Build history of the part. All positions in model axes, mm. Round coordinates to 2 decimals unless told otherwise and drop trailing zeros. Loops run counter-clockwise (first coordinate to the right, second up) from the corner with the lowest first, then second, coordinate; pieces in that order, holes last. Notation, with made-up numbers: (-21, -2) - (-12, -2) arc R15 cw to (-12, 2) - close; hole circle Ø7 at (-7, 43.25). An arc over 180 degrees is marked (long way). Put each result on its own line as item: value. Start each with the question number.
from build123d import *

# Parameters (mm, degrees)
SKETCH_1_R      = 5
EXTRUDE_1_DEPTH = 185
SKETCH_2_R      = 4
EXTRUDE_2_DEPTH = 8
CHAMFER_1_SIZE  = 0.5


with BuildPart() as part:
    # 草图1 → 凸台-拉伸1 (new body)
    with BuildSketch(Plane.XY):
        Circle(SKETCH_1_R)
    extrude(amount=EXTRUDE_1_DEPTH)

    # 草图2 → 凸台-拉伸2 (add)
    with BuildSketch(Plane(origin=(0, 0, 0), x_dir=(-1, 0, 0), z_dir=(0, 0, -1))):
        with Locations(Location((0, 0, 0), (0, 0, 180))):
            Circle(SKETCH_2_R)
    extrude(amount=EXTRUDE_2_DEPTH)

    # 倒角1
    chamfer_1_edges = [part.edges().sort_by_distance(p)[0] for p in [
        (-5, 0, 185),
        (-4, 0, -8),
    ]]
    chamfer(chamfer_1_edges, length=CHAMFER_1_SIZE)


solid = part.part
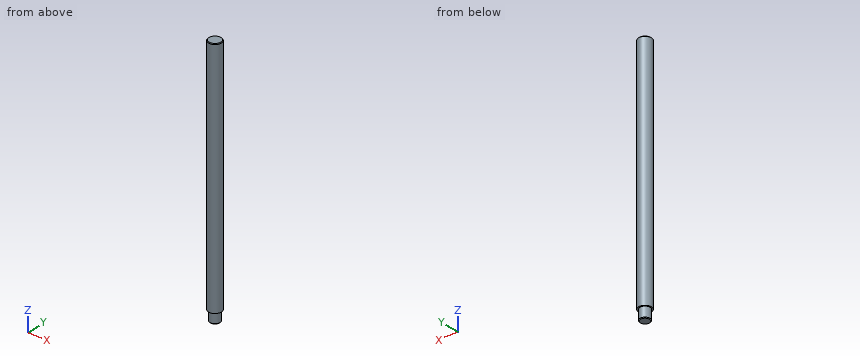
Item 1: Drop flat-ended pins along their axis: pin 1 Ø5 at (x, z) = (-3, 67) entering from -Y; pin 2 Ø4 at (y, z) = (2.5, 132) entering from +X. Give the stop position or say it passes through.
Item 2: Drill centre lines: probe 1 along Y at (x, z) = (0.25, 23); probe 2 along X at (y, z) = (-3, 38.5); probe 3 along X at (y, z) = (-2.25, 118). Where is each one in solid material? Low to high. Write a range as [from, to].
Item 3: Slice it at A-A (z = 134.5). Give the cut face in (x, y).
Computed values:
1. pin 1: stops at y = -4.97
1. pin 2: stops at x = 4.97
2. probe 1: y = [-4.99, 4.99]
2. probe 2: x = [-4, 4]
2. probe 3: x = [-4.47, 4.47]
3. outline: circle Ø10 at (0, 0)
